Can you work these out from the model? Positions are in its coordinate system, mm. Coordinates: 2 decimals unless noted, no trailing zeros. Write each loop counter-clockwise with the first axis right and the second up, starting at its lowest first coordinate (ties: lowest second). Pieces come first, ordered by that corner, then holes.
```python
from build123d import *

# Parameters (mm, degrees)
SKETCH_1_W      = 70
SKETCH_1_H      = 30
SKETCH_1_R      = 4.5
EXTRUDE_1_DEPTH = 10.5


with BuildPart() as part:
    # 草图1 → 凸台-拉伸1 (new body)
    with BuildSketch(Plane.XY):
        with Locations((35, 15)):
            Rectangle(SKETCH_1_W, SKETCH_1_H)
        with Locations(Location((11.5, 20, 0), (0, 0, 180))):
            Circle(SKETCH_1_R, mode=Mode.SUBTRACT)
        with Locations(Location((58.5, 9, 0), (0, 0, 180))):
            Circle(SKETCH_1_R, mode=Mode.SUBTRACT)
    extrude(amount=EXTRUDE_1_DEPTH)


solid = part.part
```
1. If we section it at A-A, the plane x = 11.5: List the corners of the cut face in (y, z) for me.
2. I'm going to push a flat-ended pin straight in: P1, Ø7, axis at x = 58.5, y = 9, coming from the +Z side. Where does the tip first touch, or does it pass through?
3. If I drill on L1, parallel to X at y = 9, z = 6.5; L2, parallel to Y at x = 11.5, z = 6; L3, parallel to Y at x = 58.5, z = 4, over which ranges is the centre line in solid material (lowest first)?
4. If we section it at B-B, the plane y = 9: List the corners of the cut face in (x, z) for me.
5. If we section it at C-C, the plane z = 8.75: List the corners of the cut face in (x, y) for me, plus the area to 3 significant figures.
Answers:
1. outline: (0, 0) - (15.5, 0) - (15.5, 10.5) - (0, 10.5) - close; (24.5, 0) - (30, 0) - (30, 10.5) - (24.5, 10.5) - close
2. P1: passes through
3. L1: x = 0 to 54, 63 to 70
3. L2: y = 0 to 15.5, 24.5 to 30
3. L3: y = 0 to 4.5, 13.5 to 30
4. outline: (0, 0) - (54, 0) - (54, 10.5) - (0, 10.5) - close; (63, 0) - (70, 0) - (70, 10.5) - (63, 10.5) - close
5. outline: (0, 0) - (70, 0) - (70, 30) - (0, 30) - close; hole circle Ø9 at (11.5, 20); hole circle Ø9 at (58.5, 9)
5. area: 1,970 mm2
